The model under review builds one solid part; all positions refer to its coordinate system, in mm. A direction names the side the tool comes from. Coordinates: 2 decimals unless noted, no trailing zeros. Order: outer loops, then holes, each group sorted by start corner. A loop starts at its lowest first (then second) coordinate and runs counter-clockwise, first axis right, second up.
```python
from build123d import *

# Parameters (mm, degrees)
SKETCH1_R           = 35.5
SKETCH1_R_2         = 25
BOSS_EXTRUDE1_DEPTH = 10
SKETCH2_R           = 1.25
CUT_EXTRUDE1_DEPTH  = 52.190819489
SKETCH3_R           = 35.5
SKETCH3_R_2         = 26.5
CUT_EXTRUDE2_DEPTH  = 2
M4_TAPPED_HOLE1_D   = 3.3
CHAMFER1_SIZE       = 1


with BuildPart() as part:
    # Sketch1 → Boss-Extrude1 (new body)
    with BuildSketch(Plane.XY):
        Circle(SKETCH1_R)
        Circle(SKETCH1_R_2, mode=Mode.SUBTRACT)
    extrude(amount=BOSS_EXTRUDE1_DEPTH)

    # Sketch2 → Cut-Extrude1 (cut, through all)
    with BuildSketch(Plane.XY.offset(10)):
        with Locations((0, 29.5)):
            Circle(SKETCH2_R)
        with Locations((29.5, 0)):
            Circle(SKETCH2_R)
        with Locations((0, -29.5)):
            Circle(SKETCH2_R)
        with Locations((-29.5, 0)):
            Circle(SKETCH2_R)
    extrude(amount=-CUT_EXTRUDE1_DEPTH, mode=Mode.SUBTRACT)

    # Sketch3 → Cut-Extrude2 (cut)
    with BuildSketch(Plane(origin=(0, 0, 0), x_dir=(-1, 0, 0), z_dir=(0, 0, -1))):
        Circle(SKETCH3_R)
        Circle(SKETCH3_R_2, mode=Mode.SUBTRACT)
    extrude(amount=-CUT_EXTRUDE2_DEPTH, mode=Mode.SUBTRACT)

    # M4 Tapped Hole1 (through all)
    with Locations(Plane.XY.offset(10)):
        with Locations((0, -29.5), (-29.5, 0), (0, 29.5), (29.5, 0)):
            Hole(M4_TAPPED_HOLE1_D / 2)

    # Chamfer1
    chamfer1_edges = [part.edges().sort_by_distance(p)[0] for p in [
        (-35.5, 0, 2),
        (-35.5, 0, 10),
    ]]
    chamfer(chamfer1_edges, length=CHAMFER1_SIZE)


solid = part.part
```
(1) We need section B-B, the plane z = 6.5. Write out the cut boundary in (x, y).
A:
outline: circle Ø71 at (0, 0); hole circle Ø3.3 at (-29.5, 0); hole circle Ø50 at (0, 0); hole circle Ø3.3 at (0, -29.5); hole circle Ø3.3 at (0, 29.5); hole circle Ø3.3 at (29.5, 0)
(2) Draft analysis for pull direction Y (two halves, no side actions). For faces 3 (the face through (10.1, 23.2, 10)), 4 (the face through (0.215, -27.864, 5.944)), 5 (the face through (-7.696, -34.656, 5.958)), state which applies: released by +Y, released by -Y, zero draft, split by the parting line, or undercut.
A:
face 3: zero draft
face 4: undercut
face 5: split by the parting line
(3) Machinability: for faces 1 (the face through (-14.246, 22.345, 0.986)), 2 (the face through (0.215, 31.136, 5.944)), which of the approach directions +Z, -Z, +X, -X, +Y, -Y give a long, thin tool a straight path to every point of the face, cutting with its end or side? Answer none if there is none.
A:
face 1: -Z
face 2: +Z, -Z
(4) Wall thickness on probe 1 along Y at (x, z) = (0, 8); probe 2 along X at (y, z) = (-0.5, 6.5) (3 decimals); probe 3 along X at (y, z) = (5, 9.25): over which ranges is each line inside the solid? List them lowest first.
A:
probe 1: y = -35.5 to -31.15, -27.85 to -25, 25 to 27.85, 31.15 to 35.5
probe 2: x = -35.496 to -31.072, -27.928 to -24.995, 24.995 to 27.928, 31.072 to 35.496
probe 3: x = -34.89 to -24.49, 24.49 to 34.89
(5) For pin 1 Ø5 at (x, z) = (1.5, 5) entering from -Y; pin 2 Ø2 at (x, z) = (17, 5.5) entering from -Y; pin 3 Ø2 at (y, z) = (8, 5) entering from -X; pin 4 Ø10 at (x, y) = (3.5, 23) entering from +Z, all flat-tipped, find the tip position at first contact; note any pin that passes through.
A:
pin 1: stops at y = -35.5
pin 2: stops at y = -31.69
pin 3: stops at x = -34.8
pin 4: stops at z = 10
(6) We need section A-A, the plane x = 0. Write out the cut boundary in (y, z).
A:
outline: (-35.5, 3) - (-34.5, 2) - (-31.15, 2) - (-31.15, 10) - (-34.5, 10) - (-35.5, 9) - close; (-27.85, 2) - (-26.5, 2) - (-26.5, 0) - (-25, 0) - (-25, 10) - (-27.85, 10) - close; (25, 0) - (26.5, 0) - (26.5, 2) - (27.85, 2) - (27.85, 10) - (25, 10) - close; (31.15, 2) - (34.5, 2) - (35.5, 3) - (35.5, 9) - (34.5, 10) - (31.15, 10) - close
